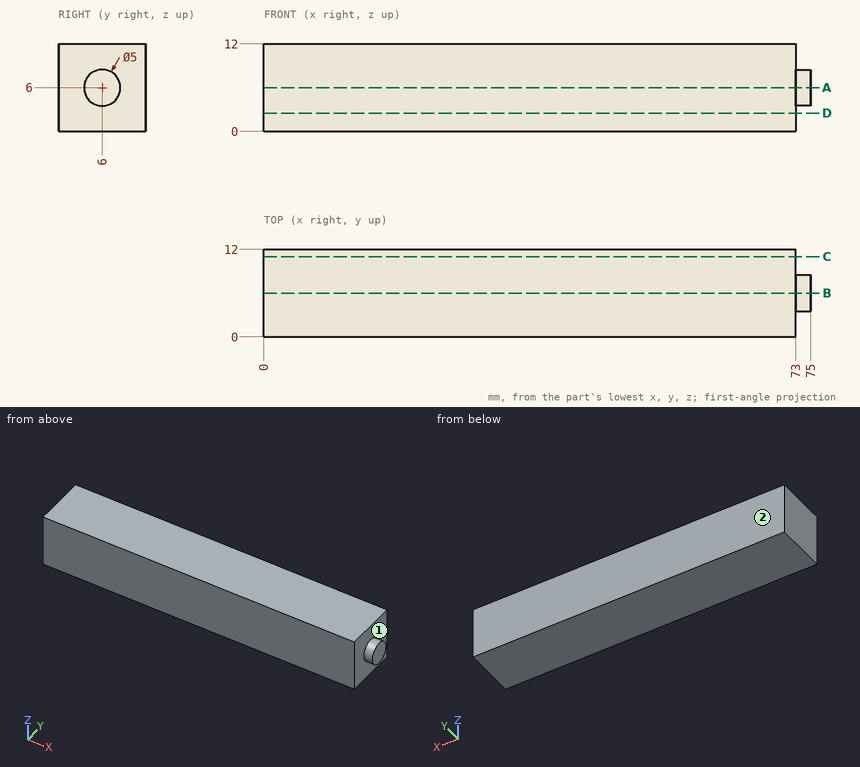
Geometry check sheet. Reference: drawing and pictorial views, mm from the part's lowest x, y, z. A direction names the side the tool comes from. Coordinates: 2 decimals unless noted, no trailing zeros. Order: outer loops, then holes, each group sorted by start corner. A loop starts at its lowest first (then second) coordinate and runs counter-clockwise, first axis right, second up. Notation, with made-up numbers: (45, 84.5) - (60, 84.5) arc R29 cw to (60, 117.5) - close; hole circle Ø7 at (22.25, -36). An arc over 180 degrees is marked (long way). Answer in a Markdown table with one row per item. Add a question column.
1) Set-up check for the marked faces 1 and 2: record each of +Z, -Z, +X, -X, +Y, -Y from which the full face is reachable in a straight line by a thin tool's end or side.
2) Material ranges on line 1 along X through (y, z) = (9, 11.5), recorded low to high. Write a range as [from, to].
3) Cross-section at A-A, the plane z = 6. Record the cut outline in (x, y).
4) Cross-section at C-C, the plane y = 11. Record the cut outline in (x, z).
Check result:
| question | item | result |
|---|---|---|
| 1 | face 1 | +X |
| 1 | face 2 | +Z, -Z, +X, -X, +Y |
| 2 | line 1 | x = [0, 73] |
| 3 | outline | (0, 0) - (73, 0) - (73, 3.5) - (75, 3.5) - (75, 8.5) - (73, 8.5) - (73, 12) - (0, 12) - close |
| 4 | outline | (0, 0) - (73, 0) - (73, 12) - (0, 12) - close |
